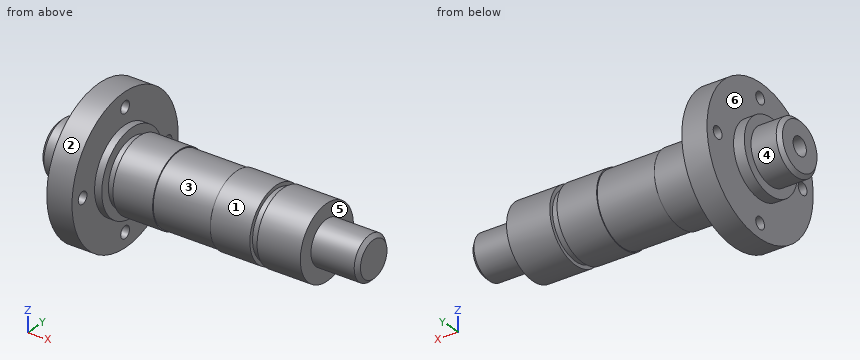
from build123d import *

# Parameters (mm, degrees)
M6_TAPPED_HOLE1_D     = 5
M6_TAPPED_HOLE1_DEPTH = 18
M6_TAPPED_HOLE1_TIP   = 1.502151548
M4_TAPPED_HOLE1_D     = 3.3
SKETCH6_W             = 2
SKETCH6_H             = 1
CHAMFER1_SIZE         = 1


with BuildPart() as part:
    # Sketch1 → Revolve1 (revolve)
    with BuildSketch(Plane.XY, mode=Mode.PRIVATE) as revolve1_sk:
        Polygon((0, 0), (87, 0), (87, 6), (74, 6), (74, 10), (62, 10), (62, 9), (60, 9), (60, 10), (49, 10), (49, 9.75), (33, 9.75), (33, 10), (20, 10), (20, 11.5), (18, 11.5), (18, 20), (11, 20), (11, 10), (8, 10), (8, 7.5), (0, 7.5), align=None)
    revolve(revolve1_sk.sketch.rotate(Axis((0, 0, 0), (1, 0, 0)), 90), axis=Axis((0, 0, 0), (1, 0, 0)))

    # M6 Tapped Hole1
    with Locations(Plane.ZY):
        with Locations((0, 0)):
            Hole(M6_TAPPED_HOLE1_D / 2, depth=M6_TAPPED_HOLE1_DEPTH)
            with Locations((0, 0, -(M6_TAPPED_HOLE1_DEPTH + M6_TAPPED_HOLE1_TIP / 2))):  # 118° drill point
                Cone(0, M6_TAPPED_HOLE1_D / 2, M6_TAPPED_HOLE1_TIP, mode=Mode.SUBTRACT)

    # M4 Tapped Hole1 (through all)
    with Locations(Plane.ZY.offset(-11)):
        with Locations((0, 16), (-16, 0), (0, -16), (16, 0)):
            Hole(M4_TAPPED_HOLE1_D / 2)

    # Sketch6 → Cut-Revolve1 (revolve, cut)
    with BuildSketch(Plane.XY, mode=Mode.PRIVATE) as cut_revolve1_sk:
        with Locations((21, 9.5)):
            Rectangle(SKETCH6_W, SKETCH6_H)
    revolve(cut_revolve1_sk.sketch.rotate(Axis((0, 0, 0), (1, 0, 0)), 90), axis=Axis((0, 0, 0), (1, 0, 0)), mode=Mode.SUBTRACT)

    # Chamfer1
    chamfer1_edges = [part.edges().sort_by_distance(p)[0] for p in [
        (87, 0, -6),
        (0, 0, -7.5),
    ]]
    chamfer(chamfer1_edges, length=CHAMFER1_SIZE)


solid = part.part
Part model, mm, in its own coordinate system. Face numbers are marked on the shaded views. A direction names the side the tool comes from. Give positions to 0.01 mm unless a question says otherwise; leave off trailing zeros. Order: outer loops, then holes, each group sorted by start corner. A loop starts at its lowest first (then second) coordinate and runs counter-clockwise, first axis right, second up. Notation, with made-up numbers: (-16.75, 35.5) - (30.25, 35.5) arc R27 ccw to (30.25, 59.5) - close; hole circle Ø1 at (61.25, 21). An arc over 180 degrees is marked (long way). Use a Markdown table: item, result.
1) Saw through at A-A on z = 16. List the corners of the cut face in (x, y), plus the area to 3 significant figures.
Checked values:
| item | result |
|---|---|
| outline | (11, -12) - (18, -12) - (18, -1.65) - (11, -1.65) - close; (11, 1.65) - (18, 1.65) - (18, 12) - (11, 12) - close |
| area | 145 mm² |
2) Two-plate mould, pull along X, no slides. Class the marked faces 3, 4, 5 and 6: +X half, -X half, draft (parallel to the pull), parting line (faces both ways), or undercut.
Checked values:
| item | result |
|---|---|
| face 3 | undercut |
| face 4 | draft |
| face 5 | +X half |
| face 6 | -X half |
3) Saw through at C-C on x = 13. List the corners of the cut face in (y, z).
Checked values:
| item | result |
|---|---|
| outline | circle Ø40 at (0, 0); hole circle Ø3.3 at (-16, 0); hole circle Ø5 at (0, 0); hole circle Ø3.3 at (0, -16); hole circle Ø3.3 at (0, 16); hole circle Ø3.3 at (16, 0) |
4) Saw through at D-D on x = 40.5. List the corners of the cut face in (y, z).
Checked values:
| item | result |
|---|---|
| outline | circle Ø19.5 at (0, 0) |
5) Probe L1, parallel to Y at x = 14, z = 0; L2, parallel to X at y = -3, z = -13; L3, parallel to X at y = 5.5, z = 7. List the from-to ranges inside material, lowest first. Write a range as from..to.
Checked values:
| item | result |
|---|---|
| L1 | -20..-17.65, -14.35..-2.5, 2.5..14.35, 17.65..20 |
| L2 | 11..18 |
| L3 | 8..74 |
6) 3-axis set-ups, long thin cutter, end or side, ignore diameter. For the marked faces 1 and 2: which of +Z, -Z, +X, -X, +Y, -Y reach the whole face in a straight line?
Checked values:
| item | result |
|---|---|
| face 1 | +X |
| face 2 | +X, -X |
7) Flat gauge pins, fed straight in: P1, Ø6, axis at x = 74.5, y = -6, coming from the +Z side; P2, Ø22, axis at y = 2, z = 3, coming from the -X side; P3, Ø8, axis at x = 70, y = -9.5, coming from the -Z side; P4, Ø2.5, axis at y = 0, z = -16, coming from the +X side. Where does each tip first touch, or does it go through?
Checked values:
| item | result |
|---|---|
| P1 | z = 9.53 |
| P2 | x = 0 |
| P3 | z = -8.35 |
| P4 | through |
